Verification items for this drawing (mm, ordinates from the low corner). Coordinates: 2 decimals unless noted, no trailing zeros. Write each loop counter-clockwise with the first axis right and the second up, starting at its lowest first coordinate (ties: lowest second). Pieces come first, ordered by that corner, then holes. Notation, with made-up numbers: (65, -24) -> (89, -24) arc R19 ccw to (89, 3) -> close; hole circle Ø7 at (8.5, -10). An arc over 180 degrees is marked (long way). One line per item, written item: value. Start each with the question number.
1) Sectioned sample at D-D on x = 225. Enter the section's corners in (y, z).
2) Gauge pin test, flat end, axial feed: P1, Ø8, axis at x = 225, y = 15, coming from the +Z side. Record the tip position at first contact, or that the pin passes through.
3) Scan lines: line 1 along Y through (x, z) = (225, 7); line 2 along X through (y, z) = (135.5, 2.25); line 3 along Y through (x, z) = (278, 8.25). Record each from-to range of solid material in increasing order. Write a range as [from, to].
4) Sectioned sample at C-C on z = 5. Enter the section's corners in (x, y), plus the area to 3 significant figures.
5) Sectioned sample at A-A on y = 15. Enter the section's corners in (x, z), plus the area to 3 significant figures.
6) Sectioned sample at B-B on x = 287. Enter the section's corners in (y, z).
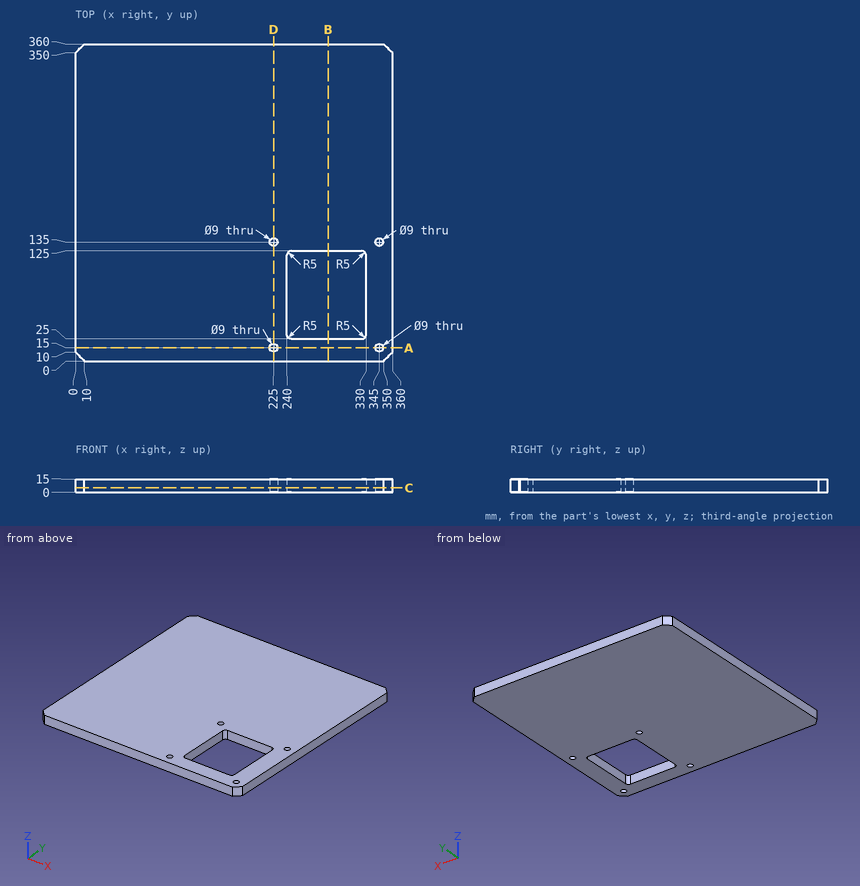
Answers:
1. outline: (0, 0) -> (10.5, 0) -> (10.5, 15) -> (0, 15) -> close; (19.5, 0) -> (130.5, 0) -> (130.5, 15) -> (19.5, 15) -> close; (139.5, 0) -> (360, 0) -> (360, 15) -> (139.5, 15) -> close
2. P1: passes through
3. line 1: y = [0, 10.5], [19.5, 130.5], [139.5, 360]
3. line 2: x = [0, 220.53], [229.47, 340.53], [349.47, 360]
3. line 3: y = [0, 25], [125, 360]
4. outline: (0, 10) -> (10, 0) -> (350, 0) -> (360, 10) -> (360, 350) -> (350, 360) -> (10, 360) -> (0, 350) -> close; hole circle Ø9 at (225, 15); hole circle Ø9 at (225, 135); hole (240, 30) arc R5 ccw to (245, 25) -> (325, 25) arc R5 ccw to (330, 30) -> (330, 120) arc R5 ccw to (325, 125) -> (245, 125) arc R5 ccw to (240, 120) -> close; hole circle Ø9 at (345, 15); hole circle Ø9 at (345, 135)
4. area: 120,000 mm2
5. outline: (0, 0) -> (220.5, 0) -> (220.5, 15) -> (0, 15) -> close; (229.5, 0) -> (340.5, 0) -> (340.5, 15) -> (229.5, 15) -> close; (349.5, 0) -> (360, 0) -> (360, 15) -> (349.5, 15) -> close
5. area: 5,130 mm2
6. outline: (0, 0) -> (25, 0) -> (25, 15) -> (0, 15) -> close; (125, 0) -> (360, 0) -> (360, 15) -> (125, 15) -> close
